from build123d import *

# Parameters (mm, degrees)
SKETCH2_R           = 10
BOSS_EXTRUDE1_DEPTH = 15


with BuildPart() as part:
    # Sketch1 → Revolve1 (revolve)
    with BuildSketch(Plane.XY, mode=Mode.PRIVATE) as revolve1_sk:
        Polygon((0, 0), (0, 410), (50, 410), (50, 210), (40, 210), (40, 60), (20, 60), (20, 0), align=None)
    revolve(revolve1_sk.sketch.rotate(Axis((0, 0, 0), (0, 1, 0)), 90), axis=Axis((0, 0, 0), (0, 1, 0)))

    # Sketch2 → Boss-Extrude1 (add, symmetric)
    with BuildSketch(Plane.XY):
        with BuildLine():
            Line((-25, 450), (-25, 410))
            Line((-25, 410), (25, 410))
            Line((25, 410), (25, 450))
            ThreePointArc((25, 450), (0, 475), (-25, 450))
        make_face()
        with Locations((0, 450)):
            Circle(SKETCH2_R, mode=Mode.SUBTRACT)
    extrude(amount=BOSS_EXTRUDE1_DEPTH, both=True)


solid = part.part
Part model, mm, in its own coordinate system. A direction names the side the tool comes from. Give positions to 0.01 mm unless a question says otherwise; leave off trailing zeros. Loops run counter-clockwise (first coordinate to the right, second up) from the corner with the lowest first, then second, coordinate; pieces in that order, holes last.
(1) Pin check, flat tips, straight feed: pin 1 (2 mm diameter, centred on x = 16, y = 324.5, fed in from -Z); pin 2 (5 mm diameter, centred on x = 26, z = -27, fed in from -Y); pin 3 (15 mm diameter, centred on x = -7.5, y = 441.5, fed in from +Z); pin 4 (12 mm diameter, centred on x = 0, y = 450, fed in from +Z). Stop position of each tip, or through.
Return value:
pin 1: stops at z = -47.7
pin 2: stops at y = 60
pin 3: stops at z = 15
pin 4: passes through
(2) Drill centre lines: line 1 along Y through (x, z) = (0, -5.25); line 2 along Y through (x, z) = (-30, 3); line 3 along Z through (x, y) = (1, 244.5). Where is each one in solid material? Low to high.
Return value:
line 1: y = 0 to 440, 460 to 475
line 2: y = 60 to 410
line 3: z = -49.99 to 49.99
(3) Band-saw the part on C-C (y = 136). Write the cut outline in (x, z).
Return value:
outline: circle Ø80 at (0, 0)
(4) Band-saw the part on D-D (z = -36). Write the cut outline in (x, y), and give its area (3 significant figures).
Return value:
outline: (-34.7, 210) - (-17.44, 210) - (-17.44, 60) - (17.44, 60) - (17.44, 210) - (34.7, 210) - (34.7, 410) - (-34.7, 410) - close
area: 19,100 mm2
(5) Band-saw the part on A-A (x = 0). Write the cut outline in (y, z), and give its area (4 significant figures).
Return value:
outline: (0, -20) - (60, -20) - (60, -40) - (210, -40) - (210, -50) - (410, -50) - (410, -15) - (440, -15) - (440, 15) - (410, 15) - (410, 50) - (210, 50) - (210, 40) - (60, 40) - (60, 20) - (0, 20) - close; (460, -15) - (475, -15) - (475, 15) - (460, 15) - close
area: 35,750 mm2
(6) 3-axis set-ups, long thin cutter, end or side, ignore diameter. For faces 4 (the flat face through (0, 436, -15)), 5 (the flat face through (-34, 210, 22)), 6 (the flat face through (25, 430, 0)), 7 (the flat face through (-25, 430, 0)): which of +Z, -Z, +X, -X, +Y, -Y reach the whole face in a straight line?
Return value:
face 4: -Z, +X, -X, +Y
face 5: -Y
face 6: +Z, -Z, +X, +Y
face 7: +Z, -Z, -X, +Y
(7) Band-saw the part on B-B (z = 0). Write the cut outline in (x, y).
Return value:
outline: (-50, 210) - (-40, 210) - (-40, 60) - (-20, 60) - (-20, 0) - (20, 0) - (20, 60) - (40, 60) - (40, 210) - (50, 210) - (50, 410) - (25, 410) - (25, 450) arc R25 ccw to (-25, 450) - (-25, 410) - (-50, 410) - close; hole circle Ø20 at (0, 450)
(8) Pull direction X, two halves, no side cores. Call faces 1 (the cylindrical face through (-1.302, 459.915, -0.21)), 2 (the cylindrical face through (-1.76, 133.95, 39.96)), 3 (the flat face through (0, 436, 15)): pulls with the +X half, pulls with the -X half, needs draft (parallel to the pull), parting line crosses it, or undercut.
Return value:
face 1: undercut
face 2: parting line crosses it
face 3: needs draft
